Work out the finished part from the listing and answer in its coordinate system (mm). A direction names the side the tool comes from. Give positions to 0.01 mm unless a question says otherwise; leave off trailing zeros. Write each loop counter-clockwise with the first axis right and the second up, starting at its lowest first coordinate (ties: lowest second). Pieces come first, ordered by that corner, then holes. Notation, with made-up numbers: (-16.75, 58.25) -> (26.25, 58.25) arc R26 cw to (26.25, 82.25) -> close; hole circle Ø8 at (-35.75, 82.25). An arc over 180 degrees is marked (long way). Use a Markdown table: item, result. Add a question column.
Q1. Consider line 1 (Y direction, x = -5, z = 0); line 2 (X direction, y = 0.5, z = 22); line 3 (Y direction, x = -75.25, z = 0). Determine where each line is inside the solid, lowest interval first.
Q2. For a pull along Z with two mould halves and no side action, classify faces 1 (the face through (-58.4, -17, 11)), 2 (the face through (-7.2, -3.8, 27.54)), 3 (the face through (-7.199, 39.923, 20.765)) as pulls with the +Z half, pulls with the -Z half, needs draft (parallel to the pull), parting line crosses it, or undercut.
Q3. Section C-C, the plane z = -37 is taken. Give the vertices of the cut face in (x, y), plus the area to 3 significant figures.
Q4. For faces 4 (the face through (-64.4, 6, 14)), 5 (the face through (-14.2, 19, 9)), 6 (the face through (-7.2, -30.62, 5.96)), determine the directions among +Z, -Z, +X, -X, +Y, -Y from which every point of the face is accessible in a straight line to the end or side of a thin tool.
Q5. Section A-A, the plane z = 0 is taken. State how many separate pieces and enclosed holes the cut face has, plus the area to 3 significant figures.
Q6. Section D-D, the plane y = 32.5 is taken. Give the vertices of the cut face in (x, z), plus the area to 3 significant figures.
Q7. Each of these flat-tipped pins is pushed along its axis until it touches: pin 1 Ø1 at (y, z) = (-31, 12.5) entering from -X; pin 2 Ø10 at (x, y) = (-77, -13.5) entering from +Z; pin 3 Ø2 at (x, z) = (-65.5, 13.5) entering from -Y; pin 4 Ø7.5 at (y, z) = (-32.5, 0) entering from -X. Where does it stop, or does it pass through?
from build123d import *

# Parameters (mm, degrees)
BOLT_HOLES_SKETCH_R             = 6.25
FLANGE_BOLT_HOLES_4X_12_5_DEPTH = 98.75295392
COUNTERBORE_SKETCH_R            = 19
COUNTERBORE_38X24_DEPTH         = 24
THROUGH_BORE_30_REACH           = 110.925
THROUGH_BORE_SKETCH_R           = 15
BORE_CHAMFER_3MM_SIZE           = 3
BORE_CHAMFER_3MM_SIZE2          = 0.18348786


with BuildPart() as part:
    # Sleeve Profile Sketch → Flanged Sleeve Body (revolve)
    with BuildSketch(Plane.XY, mode=Mode.PRIVATE) as flanged_sleeve_body_sk:
        Polygon((0, 0), (0, 45), (-14.2, 45), (-14.2, 20), (-58.4, 20), (-58.4, 25), (-88.4, 25), (-88.4, 0), align=None)
    revolve(flanged_sleeve_body_sk.sketch.rotate(Axis((-88.4, 0, 0), (1, 0, 0)), 90), axis=Axis((-88.4, 0, 0), (1, 0, 0)))

    # Bolt Holes Sketch → Flange Bolt Holes 4xØ12.5 (cut, through all)
    with BuildSketch(Plane.ZY.offset(14.2)):
        with Locations((0, -32.5)):
            Circle(BOLT_HOLES_SKETCH_R)
        with Locations((-32.5, 0)):
            Circle(BOLT_HOLES_SKETCH_R)
        with Locations((0, 32.5)):
            Circle(BOLT_HOLES_SKETCH_R)
        with Locations((32.5, 0)):
            Circle(BOLT_HOLES_SKETCH_R)
    extrude(amount=-FLANGE_BOLT_HOLES_4X_12_5_DEPTH, mode=Mode.SUBTRACT)

    # Counterbore Sketch → Counterbore Ø38x24 (cut)
    with BuildSketch(Plane.ZY.offset(88.4)):
        Circle(COUNTERBORE_SKETCH_R)
    extrude(amount=-COUNTERBORE_38X24_DEPTH, mode=Mode.SUBTRACT)

    # Through Bore Sketch → Through Bore Ø30 (cut, up to next)
    with BuildSketch(Plane(origin=(0, 0, 0), x_dir=(0, 0, -1), z_dir=(1, 0, 0)), mode=Mode.PRIVATE) as through_bore_30_sk1:
        Circle(THROUGH_BORE_SKETCH_R)
    through_bore_30_tool1 = extrude(through_bore_30_sk1.sketch, amount=-THROUGH_BORE_30_REACH, mode=Mode.PRIVATE) & part.part
    add(through_bore_30_tool1.solids().sort_by_distance((0, 0, 0))[0], mode=Mode.SUBTRACT)

    # Bore Chamfer 3mm
    bore_chamfer_3mm_edges = [part.edges().sort_by_distance(p)[0] for p in [
        (0, 0, 15),
    ]]
    bore_chamfer_3mm_side = [part.faces().sort_by_distance(p)[0] for p in [
        (0, 0, -43.727207794),
    ]]
    chamfer(bore_chamfer_3mm_edges, length=BORE_CHAMFER_3MM_SIZE, length2=BORE_CHAMFER_3MM_SIZE2, reference=bore_chamfer_3mm_side[0])


solid = part.part
Result set:
| question | item | result |
|---|---|---|
| 1 | line 1 | y = -45 to -38.75, -26.25 to -15, 15 to 26.25, 38.75 to 45 |
| 1 | line 2 | x = -88.4 to -58.4, -14.2 to 0 |
| 1 | line 3 | y = -25 to -19, 19 to 25 |
| 2 | face 1 | needs draft |
| 2 | face 2 | undercut |
| 2 | face 3 | parting line crosses it |
| 3 | outline | (-14.2, -25.61) -> (0, -25.61) -> (0, -4.34) -> (-14.2, -4.34) -> close; (-14.2, 4.34) -> (0, 4.34) -> (0, 25.61) -> (-14.2, 25.61) -> close |
| 3 | area | 604 mm2 |
| 4 | face 4 | -X |
| 4 | face 5 | none |
| 4 | face 6 | +X, -X |
| 5 | separate pieces | 4 |
| 5 | enclosed holes | 0 |
| 5 | area | 1,350 mm2 |
| 6 | outline | (-14.2, -31.12) -> (0, -31.12) -> (0, -6.25) -> (-14.2, -6.25) -> close; (-14.2, 6.25) -> (0, 6.25) -> (0, 31.12) -> (-14.2, 31.12) -> close |
| 6 | area | 706 mm2 |
| 7 | pin 1 | stops at x = -14.2 |
| 7 | pin 2 | stops at z = 23.51 |
| 7 | pin 3 | stops at y = -21.65 |
| 7 | pin 4 | passes through |
